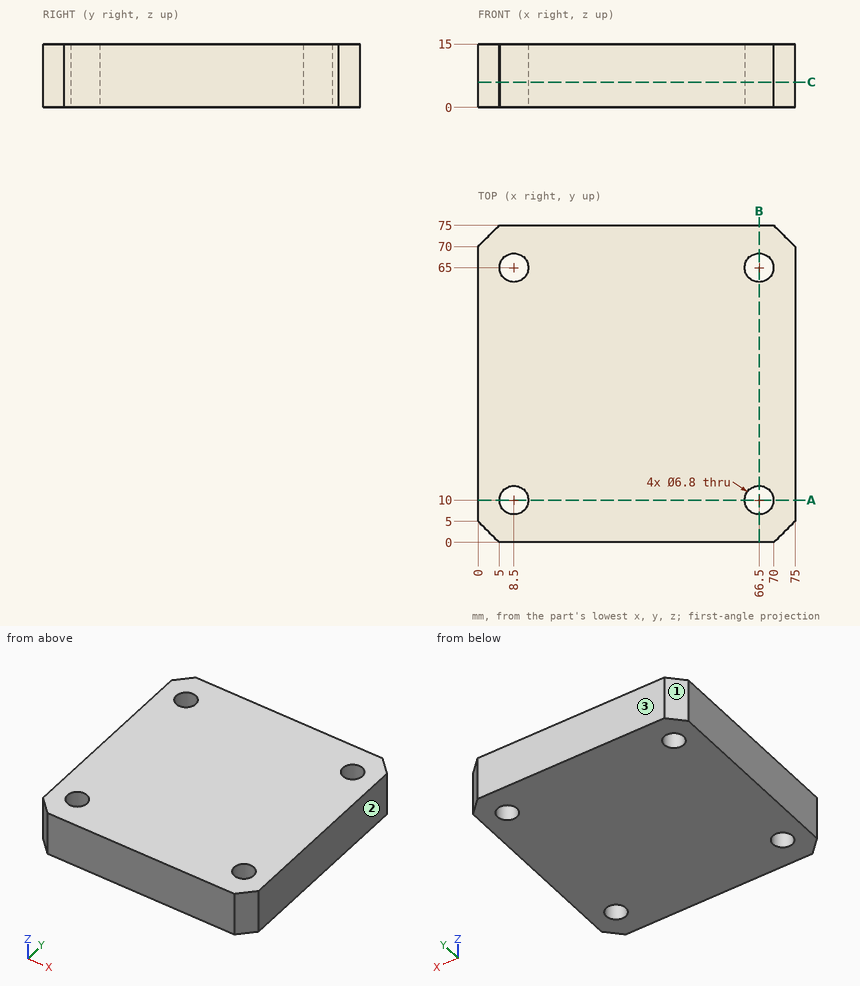
For this review, use the dimensioned drawing (mm, ordinates from the lowest corner) and the shaded views. Round coordinates to 2 decimals unless told otherwise and drop trailing zeros. Write each loop counter-clockwise with the first axis right and the second up, starting at its lowest first coordinate (ties: lowest second). Pieces come first, ordered by that corner, then holes. Notation, with made-up numbers: M 41.25,-30.75 L 52.25,-30.75 A19 cw 52.25,-4.75 Z; hole C 14.25,55.5 d8. An arc over 180 degrees is marked long. Write item = value, one per line. Start each with the question number.
(1) We need section C-C (z = 6). Give the boundary of the cut face in (x, y), then the cut area to 3 significant figures.
(2) We need section B-B (x = 66.5). Give the boundary of the cut face in (y, z).
(3) For line 1 along Y through (x, z) = (66.5, 9.25); line 2 along Y through (x, z) = (7, 12), list the stretches that pass through material, from the lowest coordinate up.
(4) We need section A-A (y = 10). Give the boundary of the cut face in (x, z).
(5) The part is to be moulded in two halves that separate along X. For the marked faces 1, 2 and 3, say which applies: +X half, -X half, draft (parallel to the pull), parting line (faces both ways), or undercut.
Results found:
q1.outline = M 0,5 L 5,0 L 70,0 L 75,5 L 75,70 L 70,75 L 5,75 L 0,70 Z; hole C 8.5,10 d6.8; hole C 8.5,65 d6.8; hole C 66.5,10 d6.8; hole C 66.5,65 d6.8
q1.area = 5,430 mm²
q2.outline = M 0,0 L 6.6,0 L 6.6,15 L 0,15 Z; M 13.4,0 L 61.6,0 L 61.6,15 L 13.4,15 Z; M 68.4,0 L 75,0 L 75,15 L 68.4,15 Z
q3.line_1 = 0 to 6.6, 13.4 to 61.6, 68.4 to 75
q3.line_2 = 0 to 6.95, 13.05 to 61.95, 68.05 to 75
q4.outline = M 0,0 L 5.1,0 L 5.1,15 L 0,15 Z; M 11.9,0 L 63.1,0 L 63.1,15 L 11.9,15 Z; M 69.9,0 L 75,0 L 75,15 L 69.9,15 Z
q5.face_1 = -X half
q5.face_2 = +X half
q5.face_3 = draft
